Part model, mm, in its own coordinate system. Face numbers are marked on the shaded views. A direction names the side the tool comes from. Round coordinates to 2 decimals unless told otherwise and drop trailing zeros. Write each loop counter-clockwise with the first axis right and the second up, starting at its lowest first coordinate (ties: lowest second). Pieces come first, ordered by that corner, then holes. Notation, with made-up numbers: M -14,75.5 L 38,75.5 A19 cw 38,96.5 Z; hole C -2.75,70 d8. An arc over 180 degrees is marked long. One line per question, with ' | ' between items. Start each with the question number.
1) Drop flat-ended pins along their axis: pin 1 Ø1.5 at (y, z) = (6.5, -4) entering from -X; pin 2 Ø4 at (x, z) = (20, -1.5) entering from +Y; pin 3 Ø6 at (x, y) = (15.5, -3.5) entering from -Z; pin 4 Ø1 at (x, z) = (8.5, 3.5) entering from -Y. Give the stop position or say it passes through.
2) Wall check: probe 1 along X at (y, z) = (0, -0.25); probe 2 along Y at (x, z) = (39.5, -2.25); probe 3 along Y at (x, z) = (39.5, 1.75). Give the ranges that are in metal, low to high. Write a range as [from, to].
3) Saw through at C-C (x = 39.5). List the corners of the cut face in (y, z).
4) Tool access for the marked faces 1 and 2: list every direction of +Z, -Z, +X, -X, +Y, -Y with a clear straight run to the whole face (end or side of a thin tool).
5) Saw through at D-D (x = 10.5). List the corners of the cut face in (y, z), plus the area to 3 significant figures.
6) Saw through at B-B (z = 0). List the corners of the cut face in (x, y).
7) Saw through at A-A (y = 0). List the corners of the cut face in (x, z).
```python
from build123d import *

# Parameters (mm, degrees)
CUT_EXTRUDE1_DEPTH      = 46.803929962
CUT_EXTRUDE1_DEPTH_BACK = 46.803929962
SKETCH2_R               = 1.6
FILLET1_R               = 0.6
CHAMFER1_SIZE           = 2
CHAMFER1_SIZE2          = 1.154700538


with BuildPart() as part:
    # Sketch1 → Base-Revolve (revolve)
    with BuildSketch(Plane.XY, mode=Mode.PRIVATE) as base_revolve_sk:
        Polygon((0, 0), (44, 0), (44, 5), (4, 5), (4, 9), (1, 9), (0, 8), align=None)
    revolve(base_revolve_sk.sketch.rotate(Axis((0, 0, 0), (-1, 0, 0)), 90), axis=Axis((0, 0, 0), (-1, 0, 0)))

    # Sketch2 → Cut-Extrude1 (cut, two sides: drawn at the far end of the back side and taken through both)
    with BuildSketch(Plane.XY.offset(-CUT_EXTRUDE1_DEPTH_BACK)):
        with Locations((39.5, 0)):
            Circle(SKETCH2_R)
    extrude(amount=CUT_EXTRUDE1_DEPTH + CUT_EXTRUDE1_DEPTH_BACK, mode=Mode.SUBTRACT)

    # Fillet1
    fillet1_edges = [part.edges().sort_by_distance(p)[0] for p in [
        (4, 0, 5),
    ]]
    fillet(fillet1_edges, radius=FILLET1_R)

    # Chamfer1
    chamfer1_edges = [part.edges().sort_by_distance(p)[0] for p in [
        (44, 0, 5),
    ]]
    chamfer1_side = [part.faces().sort_by_distance(p)[0] for p in [
        (24.3, 0, 5),
    ]]
    chamfer(chamfer1_edges, length=CHAMFER1_SIZE, length2=CHAMFER1_SIZE2, reference=chamfer1_side[0])


solid = part.part
```
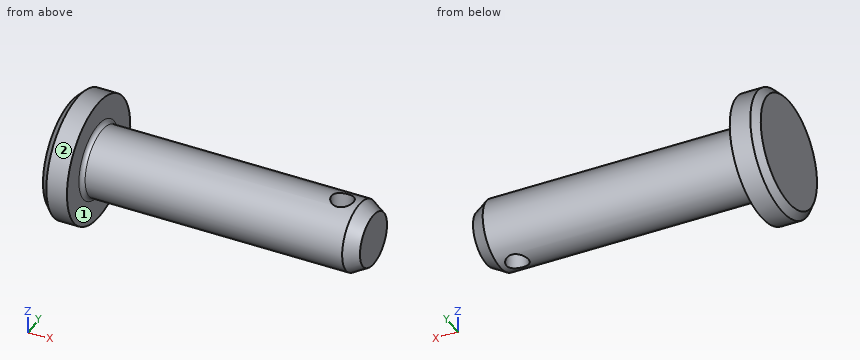
Answer key:
1) pin 1: stops at x = 0 | pin 2: stops at y = 5 | pin 3: stops at z = -4.97 | pin 4: stops at y = -4
2) probe 1: x = [0, 37.9], [41.1, 44] | probe 2: y = [-4.47, -1.6], [1.6, 4.47] | probe 3: y = [-4.68, -1.6], [1.6, 4.68]
3) outline: M -1.6,-4.74 L -1.6,4.74 A5 ccw Z; M 1.6,-4.74 A5 ccw 1.6,4.74 Z
4) face 1: +X | face 2: +X, -X
5) outline: C 0,0 d10 | area: 78.5 mm2
6) outline: M 0,-8 L 1,-9 L 4,-9 L 4,-5.6 A0.6 cw 4.6,-5 L 42,-5 L 44,-3.85 L 44,3.85 L 42,5 L 4.6,5 A0.6 cw 4,5.6 L 4,9 L 1,9 L 0,8 Z; hole C 39.5,0 d3.2
7) outline: M 0,-8 L 1,-9 L 4,-9 L 4,-5.6 A0.6 cw 4.6,-5 L 37.9,-5 L 37.9,5 L 4.6,5 A0.6 cw 4,5.6 L 4,9 L 1,9 L 0,8 Z; M 41.1,-5 L 42,-5 L 44,-3.85 L 44,3.85 L 42,5 L 41.1,5 Z
